Source: three-view drawing plus pictorial views. Frame: mm from the lowest corner of the part. Coordinates: 2 decimals unless noted, no trailing zeros. Order: outer loops, then holes, each group sorted by start corner. A loop starts at its lowest first (then second) coordinate and runs counter-clockwise, first axis right, second up. Notation, with made-up numbers: (13, -24) - (39, -24) arc R7 ccw to (39, -16) - close; hole circle Ø5 at (38.5, 22.25). An arc over 180 degrees is marked (long way). One line per question, with ' | ' between items.
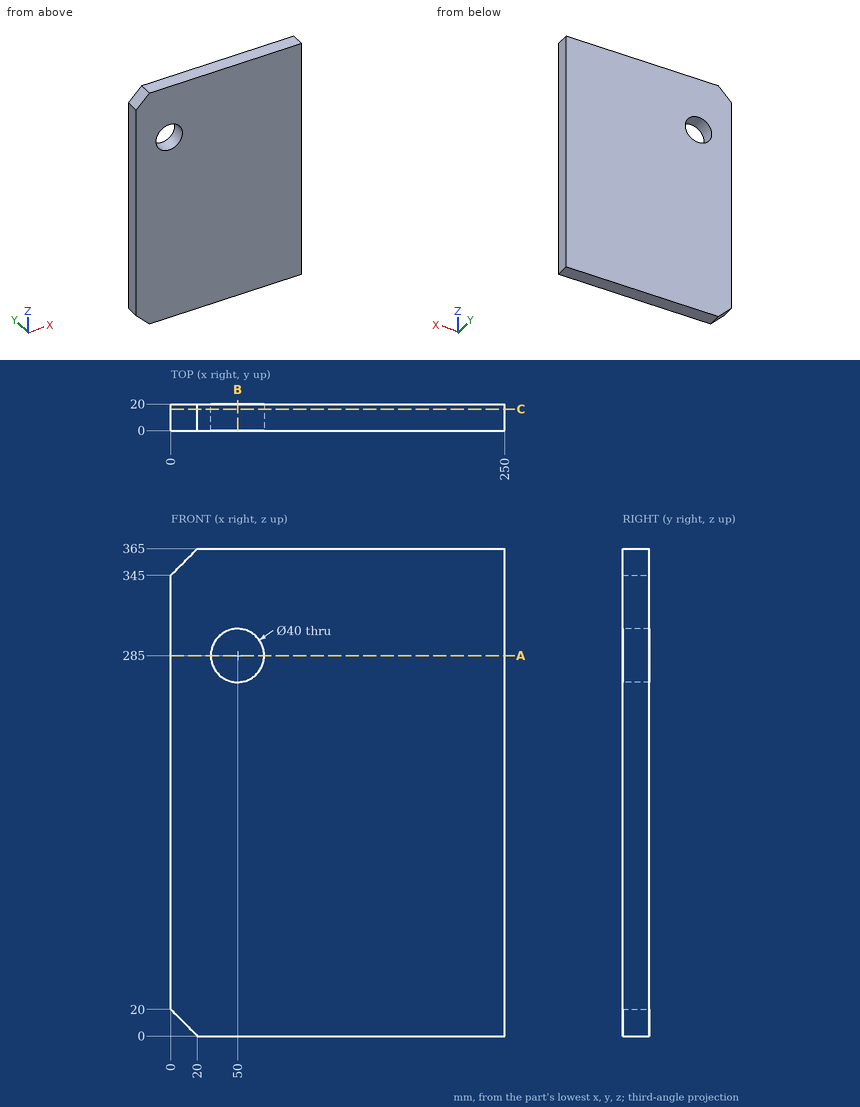
Item 1: Section B-B on x = 50. Return the cut outline in (y, z).
Data:
outline: (0, 0) - (20, 0) - (20, 265) - (0, 265) - close; (0, 305) - (20, 305) - (20, 365) - (0, 365) - close
Item 2: Section A-A on z = 285. Return the cut outline in (x, y).
Data:
outline: (0, 0) - (30, 0) - (30, 20) - (0, 20) - close; (70, 0) - (250, 0) - (250, 20) - (70, 20) - close
Item 3: Section C-C on y = 16.25. Return the cut outline in (x, z), and give its area (3 significant figures).
Data:
outline: (0, 20) - (20, 0) - (250, 0) - (250, 365) - (20, 365) - (0, 345) - close; hole circle Ø40 at (50, 285) | area: 89,600 mm^2
Item 4: Contact query for a flat-ended pin moving along its axis: P1, Ø2, axis at y = 3, z = 264.5, coming from the -X side. Output: stop coordinate, or through.
Data:
P1: x = 0
Item 5: Ray query, line 1 (Z direction, x = 50, y = 12.25); line 2 (X direction, y = 8, z = 285); line 3 (Z direction, x = 36, y = 9.25). Return the intervals inside material, ascending.
Data:
line 1: 0 to 265, 305 to 365 | line 2: 0 to 30, 70 to 250 | line 3: 0 to 270.72, 299.28 to 365
